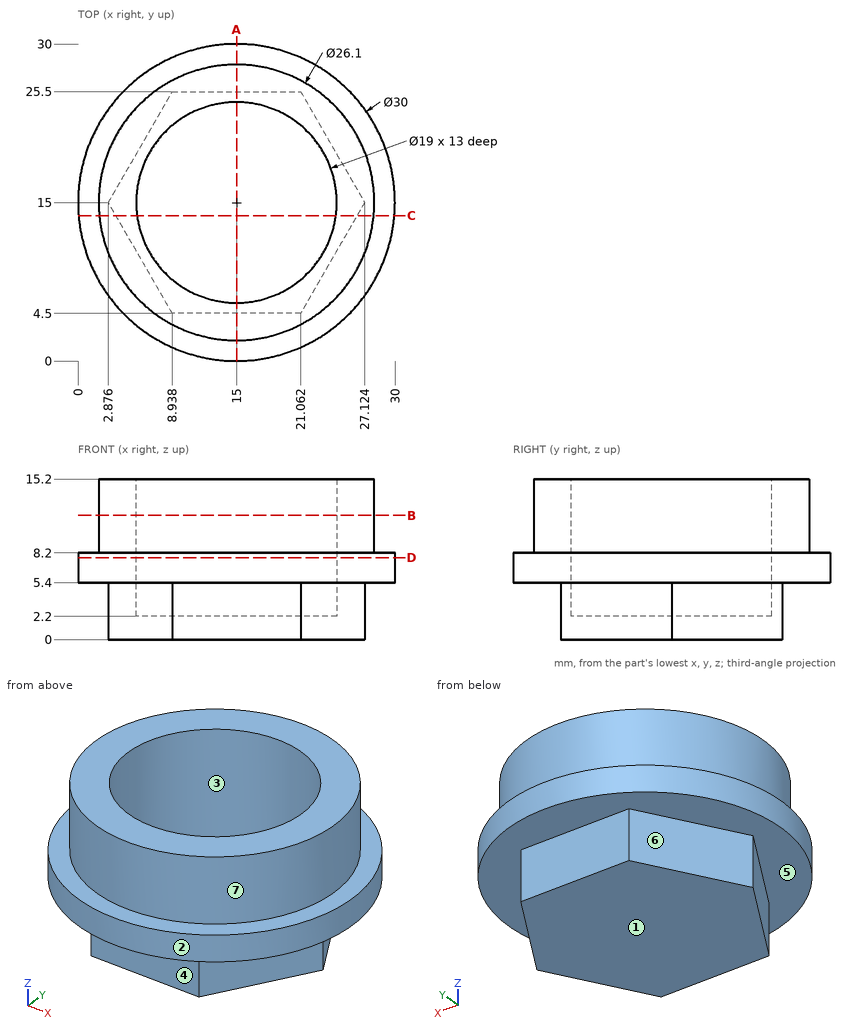
The drawing under review shows one solid part. Ordinate dimensions are in mm from its lowest x, y, z. A direction names the side the tool comes from. Round coordinates to 2 decimals unless told otherwise and drop trailing zeros. Order: outer loops, then holes, each group sorted by start corner. A loop starts at its lowest first (then second) coordinate and runs counter-clockwise, first axis right, second up. Notation, with made-up numbers: (-12, -29.5) -> (37, -29.5) arc R19 ccw to (37, -11.5) -> close; hole circle Ø2 at (30, 42.5). An arc over 180 degrees is marked (long way). Use a Markdown table: item, result.
Q1. For line 1 (Y direction, x = 15, z = 10.75); line 2 (Y direction, x = 21, z = 1.75); line 3 (Z direction, x = 17.75, y = 2.5), list the stretches that pass through material, from the lowest coordinate up.
Values:
| item | result |
|---|---|
| line 1 | y = 1.95 to 5.5, 24.5 to 28.05 |
| line 2 | y = 4.5 to 25.5 |
| line 3 | z = 5.4 to 15.2 |
Q2. Tool access review of the marked faces 4, 5, 6 and 7: name each direction out of +Z, -Z, +X, -X, +Y, -Y from which nothing blocks a thin tool from reaching the whole face with its end or side.
Values:
| item | result |
|---|---|
| face 4 | -Z, +X, -X, -Y |
| face 5 | -Z |
| face 6 | -Z, -X, +Y |
| face 7 | +Z |
Q3. Clearance check with flat-ended pins moving along their axes: P1, Ø1, axis at x = 15, z = 11, coming from the -Y side; P2, Ø15, axis at x = 15.5, y = 14, coming from the +Z side; P3, Ø2.5, axis at x = 12.5, z = 3, coming from the -Y side. State where each tip first meets the part, or that it passes through.
Values:
| item | result |
|---|---|
| P1 | stops at y = 1.95 |
| P2 | stops at z = 2.2 |
| P3 | stops at y = 4.5 |
Q4. We need section D-D on z = 7.75. Write out the cut boundary in (x, y).
Values:
| item | result |
|---|---|
| outline | circle Ø30 at (15, 15); hole circle Ø19 at (15, 15) |
Q5. We need section C-C on y = 13.75. Write out the cut boundary in (x, z).
Values:
| item | result |
|---|---|
| outline | (0.05, 5.4) -> (3.6, 5.4) -> (3.6, 0) -> (26.4, 0) -> (26.4, 5.4) -> (29.95, 5.4) -> (29.95, 8.2) -> (27.99, 8.2) -> (27.99, 15.2) -> (24.42, 15.2) -> (24.42, 2.2) -> (5.58, 2.2) -> (5.58, 15.2) -> (2.01, 15.2) -> (2.01, 8.2) -> (0.05, 8.2) -> close |
Q6. Mouldability with a two-part tool opening along Y and no side actions: class the marked faces 1, 2 and 3 as +Y half, -Y half, draft (parallel to the pull), parting line (faces both ways), or undercut.
Values:
| item | result |
|---|---|
| face 1 | draft |
| face 2 | parting line |
| face 3 | undercut |
Q7. We need section B-B on z = 11.75. Write out the cut boundary in (x, y).
Values:
| item | result |
|---|---|
| outline | circle Ø26.1 at (15, 15); hole circle Ø19 at (15, 15) |
Q8. We need section A-A on x = 15. Write out the cut boundary in (y, z).
Values:
| item | result |
|---|---|
| outline | (0, 5.4) -> (4.5, 5.4) -> (4.5, 0) -> (25.5, 0) -> (25.5, 5.4) -> (30, 5.4) -> (30, 8.2) -> (28.05, 8.2) -> (28.05, 15.2) -> (24.5, 15.2) -> (24.5, 2.2) -> (5.5, 2.2) -> (5.5, 15.2) -> (1.95, 15.2) -> (1.95, 8.2) -> (0, 8.2) -> close |
